from build123d import *

# Parameters (mm, degrees)
SKETCH1_R                = 4.3
BOSS_EXTRUDE1_DEPTH      = 6
SKETCH2_R                = 2
BOSS_EXTRUDE2_DEPTH      = 6
CHAMFER1_SIZE            = 0.2
F_3_0_3_DIAMETER_HOLE1_D = 3


with BuildPart() as part:
    # Sketch1 → Boss-Extrude1 (new body)
    with BuildSketch(Plane.XY):
        Circle(SKETCH1_R)
    extrude(amount=BOSS_EXTRUDE1_DEPTH)

    # Sketch2 → Boss-Extrude2 (add)
    with BuildSketch(Plane.XY.offset(6)):
        Circle(SKETCH2_R)
    extrude(amount=BOSS_EXTRUDE2_DEPTH)

    # Chamfer1
    chamfer1_edges = [part.edges().sort_by_distance(p)[0] for p in [
        (-4.3, 0, 0),
        (-4.3, 0, 6),
        (-2, 0, 12),
    ]]
    chamfer(chamfer1_edges, length=CHAMFER1_SIZE)

    # Ø3.0 (3) Diameter Hole1 (through all)
    with Locations(Plane(origin=(0, 5, 0), x_dir=(1, 0, 0), z_dir=(0, 1, 0))):
        with Locations((0, -3)):
            Hole(F_3_0_3_DIAMETER_HOLE1_D / 2)


solid = part.part
Could you check a few things on this model? Use its own coordinates, in mm. A direction names the side the tool comes from. Give positions to 0.01 mm unless a question says otherwise; leave off trailing zeros. Order: outer loops, then holes, each group sorted by start corner. A loop starts at its lowest first (then second) coordinate and runs counter-clockwise, first axis right, second up. Notation, with made-up numbers: (73.25, 61.25) - (88.25, 61.25) arc R13 cw to (88.25, 80.25) - close; hole circle Ø6 at (53, 18). An arc over 180 degrees is marked (long way). Return JSON: item names as keys, results as strings. Group by question number.
Q1. Suppose I cut it at B-B, the plane y = 0. Please give me the cut outline in (x, z).
Q2. Please list where these lines run through material, in increasing order: line 1 along Z through (x, y) = (0, -1.75); line 2 along Z through (x, y) = (-1, -0.5); line 3 along X through (y, z) = (3, 2.5). Write a range as [from, to].
Q3. Will these pins go through, and if not, where does the flat tip stop? pin 1 Ø4 at (x, z) = (2, 7) entering from -Y; pin 2 Ø5 at (y, z) = (1.5, 5) entering from +X.
Q4. Thinking about a two-plate mould opening in X: for faces 3 (the face through (-1, -2, 6)), 4 (the face through (0.195, -0.06, 1.513)), 5 (the face through (1.984, -3.815, 2.961)), which applies, pulls with the +X half, pulls with the -X half, needs draft (parallel to the pull), parting line crosses it, or undercut?
Q5. Suppose I cut it at D-D, the plane z = 3. Please give me the cut outline in (x, y), and give its area (3 significant figures).
Q6. Which directions (+Z, -Z, +X, -X, +Y, -Y) give clear straight access to the entire face, cutting with the end or side of a thin tool? Please do faces 1 (the face through (0, -2, 9)), 2 (the face through (0, 0, 12)).
Q7. Suppose I cut it at A-A, the plane x = 0. Please give me the cut outline in (y, z), and give its area (3 significant figures).
Q8. Suppose I cut it at C-C, the plane z = 4.75. Please give me the cut outline in (x, y), and give its area (3 significant figures).
Resolved:
{
 "1": {"outline": "(-4.3, 0.2) - (-4.1, 0) - (4.1, 0) - (4.3, 0.2) - (4.3, 5.8) - (4.1, 6) - (2, 6) - (2, 11.8) - (1.8, 12) - (-1.8, 12) - (-2, 11.8) - (-2, 6) - (-4.1, 6) - (-4.3, 5.8) - close; hole circle Ø3 at (0, 3)"},
 "2": {"line 1": "z = [0, 1.5], [4.5, 12]", "line 2": "z = [0, 1.88], [4.12, 12]", "line 3": "x = [-3.08, -1.41], [1.41, 3.08]"},
 "3": {"pin 1": "stops at y = -4.28", "pin 2": "stops at x = 4.3"},
 "4": {"face 3": "needs draft", "face 4": "undercut", "face 5": "parting line crosses it"},
 "5": {"outline": "(-1.5, -4.03) - (-1.5, 4.03) arc R4.3 ccw to start; (1.5, -4.03) arc R4.3 ccw to (1.5, 4.03) - close", "area": "32.8 mm2"},
 "6": {"face 1": "+Z", "face 2": "+Z, +X, -X, +Y, -Y"},
 "7": {"outline": "(-4.3, 0.2) - (-4.1, 0) - (4.1, 0) - (4.3, 0.2) - (4.3, 1.5) - (-4.3, 1.5) - close; (-4.3, 4.5) - (4.3, 4.5) - (4.3, 5.8) - (4.1, 6) - (2, 6) - (2, 11.8) - (1.8, 12) - (-1.8, 12) - (-2, 11.8) - (-2, 6) - (-4.1, 6) - (-4.3, 5.8) - close", "area": "49.7 mm2"},
 "8": {"outline": "circle Ø8.6 at (0, 0)", "area": "58.1 mm2"}
}
